```python
from build123d import *

# Parameters (mm, degrees)
SKETCH1_R           = 5
BOSS_EXTRUDE1_DEPTH = 2.5
SKETCH2_W           = 30
SKETCH2_H           = 10
BOSS_EXTRUDE2_DEPTH = 5


with BuildPart() as part:
    # Sketch1 → Boss-Extrude1 (new, symmetric)
    with BuildSketch(Plane.XY):
        with BuildLine():
            Line((15, 0), (-15, 0))
            Line((-15, 0), (-9.925067247, 41.221900218))
            ThreePointArc((-9.925067247, 41.221900218), (0, 50), (9.925067247, 41.221900218))
            Line((9.925067247, 41.221900218), (15, 0))
        make_face()
        with Locations((0, 40)):
            Circle(SKETCH1_R, mode=Mode.SUBTRACT)
    extrude(amount=BOSS_EXTRUDE1_DEPTH, both=True)

    # Sketch2 → Boss-Extrude2 (add)
    with BuildSketch(Plane.XY.offset(2.5)):
        with Locations((0, -5)):
            Rectangle(SKETCH2_W, SKETCH2_H)
    extrude(amount=-BOSS_EXTRUDE2_DEPTH)


solid = part.part
```
Geometry check sheet. Reference: the model listing, model coordinates, mm. Coordinates: 2 decimals unless noted, no trailing zeros. Order: outer loops, then holes, each group sorted by start corner. A loop starts at its lowest first (then second) coordinate and runs counter-clockwise, first axis right, second up. Notation, with made-up numbers: M -13.5,87.5 L 33.5,87.5 A10 cw 33.5,99.5 Z; hole C 4.25,87.25 d8. An arc over 180 degrees is marked long. Answer as a JSON object with one key per item and string values.
Q1. Cross-section at D-D on x = 8.5. Record the cut outline in (y, z).
Results are:
{"outline": "M -10,-2.5 L 45.27,-2.5 L 45.27,2.5 L -10,2.5 Z"}
Q2. Cross-section at B-B on x = 0. Record the cut outline in (y, z).
Results are:
{"outline": "M -10,-2.5 L 35,-2.5 L 35,2.5 L -10,2.5 Z; M 45,-2.5 L 50,-2.5 L 50,2.5 L 45,2.5 Z"}
Q3. Cross-section at C-C on y = 40. Record the cut outline in (x, z), and give its area (3 significant figures).
Results are:
{"outline": "M -10.08,-2.5 L -5,-2.5 L -5,2.5 L -10.08,2.5 Z; M 5,-2.5 L 10.08,-2.5 L 10.08,2.5 L 5,2.5 Z", "area": "50.8 mm²"}
Q4. Release check for a two-part mould opening along Y. For faces 1 (the flat face through (-12.5, 20.3, 0)), 2 (the cylindrical face through (-0.651, 44.957, -0.035)), 3 (the flat face through (0, 14, 2.5)) record: released by +Y, released by -Y, zero draft, split by the parting line, or undercut.
Results are:
{"face 1": "released by +Y", "face 2": "undercut", "face 3": "zero draft"}
Q5. Scan lines: line 1 (Y direction, x = 0, z = 1); line 2 (X direction, y = 37, z = 0.8); line 3 (X direction, y = 30, z = -1.6). Record each from-to range of solid material in increasing order.
Results are:
{"line 1": "y = -10 to 35, 45 to 50", "line 2": "x = -10.44 to -4, 4 to 10.44", "line 3": "x = -11.31 to 11.31"}
Q6. Depth check by flat-ended pin: pin 1 Ø1.5 at (y, z) = (2.5, 0.5) entering from -X; pin 2 Ø3 at (x, z) = (0.5, 0) entering from +Y; pin 3 Ø9 at (x, y) = (0, 40) entering from -Z. Enter the tip coordinate at first touch or a pass-through.
Results are:
{"pin 1": "stops at x = -14.78", "pin 2": "stops at y = 50", "pin 3": "passes through"}
Q7. Cross-section at A-A on z = -0.3. Record the cut outline in (x, y), and give its area (3 significant figures).
Results are:
{"outline": "M -15,-10 L 15,-10 L 15,0 L 9.93,41.22 A10 ccw -9.93,41.22 L -15,0 Z; hole C 0,40 d10", "area": "1,380 mm²"}
